from build123d import *

# Parameters (mm, degrees)
SKETCH1_R               = 10
BOSS_EXTRUDE1_DEPTH     = 32.5
CHAMFER1_SIZE           = 0.5
M6_TAPPED_HOLE1_D       = 5
M6_TAPPED_HOLE1_DEPTH   = 15
M6_TAPPED_HOLE1_TIP     = 1.502151548
M6_TAPPED_HOLE2_D       = 5
M6_TAPPED_HOLE2_DEPTH   = 15
M6_TAPPED_HOLE2_TIP     = 1.502151548
CUT_EXTRUDE1_DEPTH      = 36.443617197
CUT_EXTRUDE1_DEPTH_BACK = 36.443617197
SKETCH8_R               = 3.5


with BuildPart() as part:
    # Sketch1 → Boss-Extrude1 (new, symmetric)
    with BuildSketch(Plane.XY):
        Circle(SKETCH1_R)
    extrude(amount=BOSS_EXTRUDE1_DEPTH, both=True)

    # Chamfer1
    chamfer1_edges = [part.edges().sort_by_distance(p)[0] for p in [
        (-10, 0, -32.5),
        (-10, 0, 32.5),
    ]]
    chamfer(chamfer1_edges, length=CHAMFER1_SIZE)

    # M6 Tapped Hole1
    with Locations(Plane.XY.offset(32.5)):
        with Locations((0, 0)):
            Hole(M6_TAPPED_HOLE1_D / 2, depth=M6_TAPPED_HOLE1_DEPTH)
            with Locations((0, 0, -(M6_TAPPED_HOLE1_DEPTH + M6_TAPPED_HOLE1_TIP / 2))):  # 118° drill point
                Cone(0, M6_TAPPED_HOLE1_D / 2, M6_TAPPED_HOLE1_TIP, mode=Mode.SUBTRACT)

    # M6 Tapped Hole2
    with Locations(Plane(origin=(0, 0, -32.5), x_dir=(-1, 0, 0), z_dir=(0, 0, -1))):
        with Locations((0, 0)):
            Hole(M6_TAPPED_HOLE2_D / 2, depth=M6_TAPPED_HOLE2_DEPTH)
            with Locations((0, 0, -(M6_TAPPED_HOLE2_DEPTH + M6_TAPPED_HOLE2_TIP / 2))):  # 118° drill point
                Cone(0, M6_TAPPED_HOLE2_D / 2, M6_TAPPED_HOLE2_TIP, mode=Mode.SUBTRACT)

    # Sketch8 → Cut-Extrude1 (cut, two sides: drawn at the far end of the back side and taken through both)
    with BuildSketch(Plane(origin=(0, 0, 0), x_dir=(1, 0, 0), z_dir=(0, 1, 0)).offset(-CUT_EXTRUDE1_DEPTH_BACK)):
        with Locations(Location((0, 0, 0), (0, 0, 270))):
            Circle(SKETCH8_R)
    extrude(amount=CUT_EXTRUDE1_DEPTH + CUT_EXTRUDE1_DEPTH_BACK, mode=Mode.SUBTRACT)


solid = part.part
Design review of the part built by this model. Coordinates are the model's own, in mm. A direction names the side the tool comes from. Round coordinates to 2 decimals unless told otherwise and drop trailing zeros. Order: outer loops, then holes, each group sorted by start corner. A loop starts at its lowest first (then second) coordinate and runs counter-clockwise, first axis right, second up.
1) Clearance check with flat-ended pins moving along their axes: pin 1 Ø8 at (y, z) = (8, -5) entering from +X; pin 2 Ø1 at (y, z) = (-4, 10) entering from +X; pin 3 Ø4 at (x, z) = (3.5, 15.5) entering from -Y. State where each tip first meets the part, or that it passes through.
The answers:
pin 1: stops at x = 9.17
pin 2: stops at x = 9.37
pin 3: stops at y = -9.89
2) Draft analysis for pull direction Y (two halves, no side actions). For faces 3 (the conical face through (0, 0, 16)), 4 (the cylindrical face through (9.54, 3, 0.45)), 5 (the flat face through (2, -2, 32.5)), 6 (the cylindrical face through (0.54, -2.44, 24.9)), state which applies: released by +Y, released by -Y, zero draft, split by the parting line, or undercut.
The answers:
face 3: undercut
face 4: split by the parting line
face 5: zero draft
face 6: undercut
3) For L1, parallel to Y at x = 0, z = -28; L2, parallel to X at y = 0.5, z = 11.5; L3, parallel to Y at x = -0.25, z = -10, list the stretches that pass through material, from the lowest coordinate up.
The answers:
L1: y = -10 to -2.5, 2.5 to 10
L2: x = -9.99 to 9.99
L3: y = -10 to 10
4) Machinability: for faces 1 (the cylindrical face through (-0.54, -2.44, -24.9)), 2 (the cylindrical face through (-3.417, -0.14, -0.759)), which of the approach directions +Z, -Z, +X, -X, +Y, -Y give a long, thin tool a straight path to every point of the face, cutting with its end or side? Answer none if there is none.
The answers:
face 1: -Z
face 2: +Y, -Y
5) Consider section C-C (z = 20). State the section outline as (x, y) points.
The answers:
outline: circle Ø20 at (0, 0); hole circle Ø5 at (0, 0)
6) Consider section A-A (z = -12). State the section outline as (x, y) points, plus the area to 3 significant figures.
The answers:
outline: circle Ø20 at (0, 0)
area: 314 mm2
7) Consider section B-B (z = 2). State the section outline as (x, y) points, plus the area to 3 significant figures.
The answers:
outline: (-2.87, -9.58) - (-2.87, 9.58) arc R10 ccw to start; (2.87, -9.58) arc R10 ccw to (2.87, 9.58) - close
area: 201 mm2
